CAD build for the part. Positions are in the model's coordinates, mm. A direction names the side the tool comes from. Give positions to 0.01 mm unless a question says otherwise; leave off trailing zeros. Write each loop counter-clockwise with the first axis right and the second up, starting at its lowest first coordinate (ties: lowest second). Pieces come first, ordered by that corner, then holes. Notation, with made-up numbers: (48, 47.25) -> (88, 47.25) arc R12 cw to (88, 62.25) -> close; hole circle Ø3 at (42.5, 79.5). An arc over 180 degrees is marked (long way). Use one line per item in the form item = value. Start each with the question number.
from build123d import *

# Parameters (mm, degrees)
VALVE_BODY_PROFILE_SKETCH_W  = 84
VALVE_BODY_PROFILE_SKETCH_H  = 46
VALVE_BODY_BLOCK_DEPTH       = 23
TOP_PORT_BOSS_SKETCH_R       = 15
TOP_PORT_BOSS_SKETCH_R_2     = 7.5
TOP_PORT_BOSS_30_DEPTH       = 8
BODY_WINDOW_SKETCH_W         = 24
BODY_WINDOW_SKETCH_H         = 36
BODY_WINDOW_CUT_24X36_DEPTH  = 60
SIDE_PORT_SKETCH_R           = 5
SIDE_PORT_THROUGH_BORE_DEPTH = 95
SKETCH4_3_R                  = 15
SKETCH4_3_R_2                = 5
SIDE_PORT_CUT_DEPTH          = 22
REAR_START                   = -22
REAR_PORT_SKETCH_W           = 46
REAR_PORT_SKETCH_H           = 46
REAR_PORT_SKETCH_R           = 15
REAR_PORT_CUT_DEPTH          = 22
FRONT_PORT_BOSS_SKETCH_R     = 15
FRONT_PORT_BOSS_SKETCH_R_2   = 7.5
FRONT_PORT_BOSS_30_DEPTH     = 8
FRONT_START                  = -61
SKETCH6_3_R                  = 7.5
FRONT_PORT_BORE_DEPTH        = 61


with BuildPart() as part:
    # Valve Body Profile Sketch → Valve Body Block (new, symmetric)
    with BuildSketch(Plane(origin=(0, 0, 0), x_dir=(1, 0, 0), z_dir=(0, 1, 0))):
        with Locations((0, 23)):
            Rectangle(VALVE_BODY_PROFILE_SKETCH_W, VALVE_BODY_PROFILE_SKETCH_H)
        Polygon((-20, 51.769982338), (20, 51.769982338), (20, 22.392939221), (20, -6.230017662), (-20, -6.230017662), (-20, 23), align=None)
    extrude(amount=VALVE_BODY_BLOCK_DEPTH, both=True)

    # Top Port Boss Sketch → Top Port Boss _30 (add)
    with BuildSketch(Plane(origin=(0, 23, 0), x_dir=(1, 0, 0), z_dir=(0, 1, 0))):
        with Locations(Location((0, 22.179634707, 0), (0, 0, 270))):
            Circle(TOP_PORT_BOSS_SKETCH_R)
        with Locations(Location((0, 22.179634707, 0), (0, 0, 270))):
            Circle(TOP_PORT_BOSS_SKETCH_R_2, mode=Mode.SUBTRACT)
    extrude(amount=TOP_PORT_BOSS_30_DEPTH)

    # Body Window Sketch → Body Window Cut 24x36 (cut)
    with BuildSketch(Plane.XY.offset(6.230017662)):
        Rectangle(BODY_WINDOW_SKETCH_W, BODY_WINDOW_SKETCH_H)
    extrude(amount=-BODY_WINDOW_CUT_24X36_DEPTH, mode=Mode.SUBTRACT)

    # Side Port Sketch → Side Port Through Bore (cut)
    with BuildSketch(Plane(origin=(42, 0, 0), x_dir=(0, 0, -1), z_dir=(1, 0, 0))):
        with Locations((24.791188033, 0)):
            Circle(SIDE_PORT_SKETCH_R)
    extrude(amount=-SIDE_PORT_THROUGH_BORE_DEPTH, mode=Mode.SUBTRACT)

    # Sketch4_3 → Side Port Cut (cut)
    # profile 1 of 2: a face of its own
    with BuildSketch(Plane(origin=(42, 0, 0), x_dir=(0, 0, -1), z_dir=(1, 0, 0))):
        Polygon((23.784682636, 23), (46, 23), (46, -23), (0, -23), (0, 23), align=None)
        with Locations((24.791188033, 0)):
            Circle(SKETCH4_3_R, mode=Mode.SUBTRACT)
    # profile 2 of 2: a face of its own
    with BuildSketch(Plane(origin=(42, 0, 0), x_dir=(0, 0, -1), z_dir=(1, 0, 0))):
        with Locations((24.791188033, 0)):
            Circle(SKETCH4_3_R_2)
    extrude(amount=-SIDE_PORT_CUT_DEPTH, mode=Mode.SUBTRACT)

    # Rear Port Sketch → Rear Port Cut (cut)
    with BuildSketch(Plane.ZY.offset(42).offset(REAR_START)):
        with Locations((-23, 0)):
            Rectangle(REAR_PORT_SKETCH_W, REAR_PORT_SKETCH_H)
        with Locations(Location((-24.791188033, 0, 0), (0, 0, 180))):
            Circle(REAR_PORT_SKETCH_R, mode=Mode.SUBTRACT)
    extrude(amount=REAR_PORT_CUT_DEPTH, mode=Mode.SUBTRACT)

    # Front Port Boss Sketch → Front Port Boss _30 (add)
    with BuildSketch(Plane.XZ.offset(23)):
        with Locations(Location((0, -21.097330719, 0), (0, 0, 90))):
            Circle(FRONT_PORT_BOSS_SKETCH_R)
        with Locations(Location((0, -21.097330719, 0), (0, 0, 270))):
            Circle(FRONT_PORT_BOSS_SKETCH_R_2, mode=Mode.SUBTRACT)
    extrude(amount=FRONT_PORT_BOSS_30_DEPTH)

    # Sketch6_3 → Front Port Bore (cut)
    with BuildSketch(Plane.XZ.offset(23).offset(FRONT_START)):
        with Locations(Location((0, -21.097330719, 0), (0, 0, 270))):
            Circle(SKETCH6_3_R)
    extrude(amount=FRONT_PORT_BORE_DEPTH, mode=Mode.SUBTRACT)


solid = part.part
1) 3-axis set-ups, long thin cutter, end or side, ignore diameter. For faces 4 (the face through (20, 5, -10)), 5 (the face through (-5, -23, -36)), 6 (the face through (-30.846, 5.745, -38.647)): which of +Z, -Z, +X, -X, +Y, -Y reach the whole face in a straight line?
2) Two-plate mould, pull along Z, no slides. Class faces 1 (the face through (0, 23, -29)), 2 (the face through (42, 4, -21)), 3 (the face through (-5.745, 26.944, -8.323)): released by +Z, released by -Z, zero draft, split by the parting line, or undercut.
3) Wall check: line 1 along X through (y, z) = (-15, -37.5); line 2 along Y through (x, z) = (36, -24.5); line 3 along Y through (x, z) = (10.5, -4.5). Give the ranges that are in metal, low to high. Write a range as from..to.
4) Cut at C-C (y = 13). Give the cut face in (x, z), and give its area (3 significant figures).
5) Cut at A-A (x = 0). Give the cut face in (y, z), and give its area (3 significant figures).
6) Cut at B-B (z = -46.5). Give the cut face in (x, y), and give its area (3 significant figures).
7) Cut at D-D (x = -19). Give the cut face in (y, z), and give its area (3 significant figures).
8) Pin check, flat tips, straight feed: pin 1 (7 mm diameter, centred on x = -2, z = -22.5, fed in from -Y); pin 2 (2 mm diameter, centred on x = -17.5, z = -11.5, fed in from +Y); pin 3 (8 mm diameter, centred on y = 24, z = -32.5, fed in from +X); pin 4 (5 mm diameter, centred on x = -24, z = -9.5, fed in from +Y). Stop position of each tip, or through.
Final values:
q1.face_4 = +X
q1.face_5 = -Y
q1.face_6 = -X
q2.face_1 = undercut
q2.face_2 = zero draft
q2.face_3 = split by the parting line
q3.line_1 = -20..-12, 12..20
q3.line_2 = -15..-4.99, 4.99..15
q3.line_3 = -23..-18, 18..23
q4.outline = (-42, -32.27) -> (-20, -32.27) -> (-20, -51.77) -> (-12, -51.77) -> (-12, 6.23) -> (-20, 6.23) -> (-20, -17.31) -> (-42, -17.31) -> close; (12, -51.77) -> (20, -51.77) -> (20, -32.27) -> (42, -32.27) -> (42, -17.31) -> (20, -17.31) -> (20, 6.23) -> (12, 6.23) -> close
q4.area = 1,590 mm^2
q5.outline = (-31, -36.1) -> (-23, -36.1) -> (-23, -51.77) -> (-18, -51.77) -> (-18, -28.6) -> (-31, -28.6) -> close; (-31, -13.6) -> (-18, -13.6) -> (-18, 6.23) -> (-23, 6.23) -> (-23, -6.1) -> (-31, -6.1) -> close; (18, -51.77) -> (23, -51.77) -> (23, -37.18) -> (31, -37.18) -> (31, -29.68) -> (23, -29.68) -> (23, -28.6) -> (18, -28.6) -> close; (18, -13.6) -> (31, -13.6) -> (31, -7.18) -> (23, -7.18) -> (23, 6.23) -> (18, 6.23) -> close
q5.area = 661 mm^2
q6.outline = (-20, -23) -> (20, -23) -> (20, 23) -> (-20, 23) -> close; hole (-12, -18) -> (12, -18) -> (12, 18) -> (-12, 18) -> close
q6.area = 976 mm^2
q7.outline = (-23, -51.77) -> (23, -51.77) -> (23, 6.23) -> (-23, 6.23) -> close; hole circle Ø10 at (0, -24.79)
q7.area = 2,590 mm^2
q8.pin_1 = through
q8.pin_2 = 23
q8.pin_3 = 20
q8.pin_4 = 7.83
